from build123d import *

# Parameters (mm, degrees)
SIDE_CUT_8_DEPTH_4_DEPTH             = 4
SIDE_CUT_8_DEPTH_4_DEPTH_BACK        = 37.492993619
SIDE_CUT_8_SKETCH_RIGHT_PLANE_R      = 4
CROSS_CUT_8_TWO_DIRECTION_DEPTH      = 4
CROSS_CUT_8_TWO_DIRECTION_DEPTH_BACK = 10
CROSS_CUT_8_SKETCH_TOP_PLANE_R       = 4


with BuildPart() as part:
    # Knob Profile Sketch → Knob Body Revolve (revolve)
    with BuildSketch(Plane(origin=(0, 0, 0), x_dir=(1, 0, 0), z_dir=(0, 1, 0))):
        with BuildLine():
            Line((0, 0), (0, 33.773937692))
            ThreePointArc((0, 33.773937692), (9.079795586, 27.617619401), (6.721394325, 16.904035207))
            ThreePointArc((6.721394325, 16.904035207), (5.475561114, 14.165497859), (6.490711985, 11.333333333))
            ThreePointArc((6.490711985, 11.333333333), (7, 10), (6.490711985, 8.666666667))
            ThreePointArc((6.490711985, 8.666666667), (5.487408857, 5.650786662), (7, 2.855394489))
            Line((7, 2.855394489), (7, 0))
            Line((7, 0), (0, 0))
        make_face()
    revolve(axis=Axis((0, 0, 0), (0, 0, -1)))

    # Side Cut _8 Sketch _Right Plane → Side Cut _8 Depth 4 (cut, two sides: drawn at the far end of the back side and taken through both)
    with BuildSketch(Plane(origin=(0, 0, 0), x_dir=(0, 0, -1), z_dir=(1, 0, 0)).offset(-SIDE_CUT_8_DEPTH_4_DEPTH_BACK)):
        with Locations((24, 0)):
            Circle(SIDE_CUT_8_SKETCH_RIGHT_PLANE_R)
    extrude(amount=SIDE_CUT_8_DEPTH_4_DEPTH + SIDE_CUT_8_DEPTH_4_DEPTH_BACK, mode=Mode.SUBTRACT)

    # Cross Cut _8 Sketch _Top Plane → Cross Cut _8 Two-Direction (cut, two sides: drawn at the far end of the back side and taken through both)
    with BuildSketch(Plane(origin=(0, 0, 0), x_dir=(1, 0, 0), z_dir=(0, 1, 0)).offset(-CROSS_CUT_8_TWO_DIRECTION_DEPTH_BACK)):
        with Locations(Location((0, 24, 0), (0, 0, 270))):
            Circle(CROSS_CUT_8_SKETCH_TOP_PLANE_R)
    extrude(amount=CROSS_CUT_8_TWO_DIRECTION_DEPTH + CROSS_CUT_8_TWO_DIRECTION_DEPTH_BACK, mode=Mode.SUBTRACT)


solid = part.part
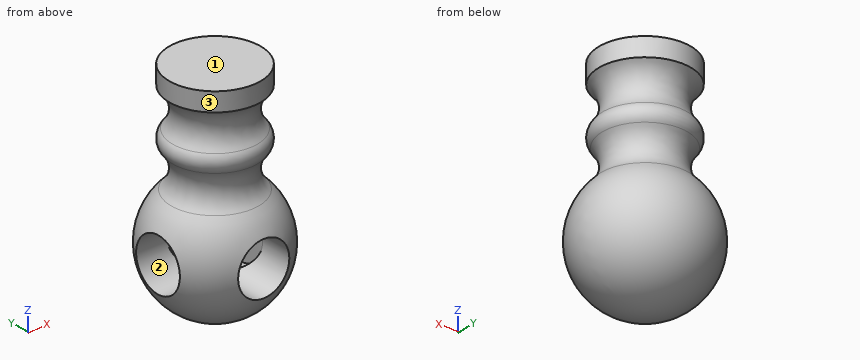
Design review of the part built by this model. Coordinates are the model's own, in mm. Face numbers are marked on the shaded views. Give positions to 0.01 mm unless a question says otherwise; leave off trailing zeros. Loops run counter-clockwise (first coordinate to the right, second up) from the corner with the lowest first, then second, coordinate; pieces in that order, holes last. Notation, with made-up numbers: (-29, 11.25) - (-21, 11.25) arc R21 cw to (-21, 34.25) - close; hole circle Ø11 at (50.25, 16.25). An arc over 180 degrees is marked (long way). Write item = value, one per line.
1) Take a section at D-D on z = -29.5. State the section outline as (x, y) points, and give its area (3 significant figures).
Result sheet:
outline = circle Ø16.16 at (0, 0)
area = 205 mm2
2) Take a section at C-C on x = 6. Count the separate pieces of the cut face and the enclosed holes in it, and give its area (3 significant figures).
Result sheet:
separate_pieces = 3
enclosed_holes = 0
area = 235 mm2
3) To check wall thickness, follow line 1 (Z direction, x = -8, y = 0.5); line 2 (Z direction, x = 0, y = -2); line 3 (Z direction, x = 6.75, y = -6.5). State the ranges of each line that lie inside material, in increasing order.
Result sheet:
line_1 = -29.59 to -27.97, -20.03 to -18.41
line_2 = -33.57 to -28, -20 to 0
line_3 = -26.78 to -21.22
4) Take a section at A-A on z = -22. State the section outline as (x, y) points.
Result sheet:
outline = (-8.92, -3.46) arc R9.57 ccw to (-3.46, -8.92) - (-3.46, -3.46) - close; (-8.92, 3.46) - (-3.46, 3.46) - (-3.46, 4) - (3.46, 4) - (3.46, 3.46) - (4, 3.46) - (4, -3.46) - (3.46, -3.46) - (3.46, -8.92) arc R9.57 ccw (long way) to start
5) Clearance check with flat-ended pins moving along their axes: pin 1 Ø1.5 at (y, z) = (7.5, -5) entering from -X; pin 2 Ø2.5 at (x, z) = (-1, -24.5) entering from -Y; pin 3 Ø1 at (x, y) = (-5.5, 4.5) entering from -Z; pin 4 Ø5 at (y, z) = (0, -24) entering from -X. State where each tip first meets the part, or that it passes through.
Result sheet:
pin_1 = through
pin_2 = 4
pin_3 = -31.2
pin_4 = 4
6) Take a section at B-B on z = -2.5. State the section outline as (x, y) points.
Result sheet:
outline = circle Ø14 at (0, 0)
7) Draft analysis for pull direction Z (two halves, no side actions). For the marked faces 1, 2 and 3, state which applies: +Z half, -Z half, draft (parallel to the pull), parting line (faces both ways), or undercut.
Result sheet:
face_1 = +Z half
face_2 = undercut
face_3 = draft
